Source: CAD feature listing. Evaluate the final solid. Frame: model axes, mm. A direction names the side the tool comes from. Give positions to 0.01 mm unless a question says otherwise; leave off trailing zeros. Loops run counter-clockwise (first coordinate to the right, second up) from the corner with the lowest first, then second, coordinate; pieces in that order, holes last.
```python
from build123d import *

# Parameters (mm, degrees)
SKETCH_1_R      = 2
EXTRUDE_1_DEPTH = 10


with BuildPart() as part:
    # 草图1 → 凸台-拉伸1 (new body)
    with BuildSketch(Plane.XY):
        with BuildLine():
            Line((0, 10), (-2.5, 10))
            Line((-2.5, 10), (-2.5, 27.142110135))
            Line((-2.5, 27.142110135), (-2.5, 28))
            Line((-2.5, 28), (2, 28))
            Line((2, 28), (2, 20))
            ThreePointArc((2, 20), (10, 12), (18, 20))
            Line((18, 20), (18, 28))
            Line((18, 28), (22.5, 28))
            Line((22.5, 28), (22.5, 10))
            Line((22.5, 10), (20, 10))
            Line((20, 10), (20, 0))
            Line((20, 0), (0, 0))
            Line((0, 0), (0, 10))
        make_face()
        with Locations((10, 5)):
            Circle(SKETCH_1_R, mode=Mode.SUBTRACT)
    extrude(amount=EXTRUDE_1_DEPTH)


solid = part.part
```
(1) First-contact query: pin 1 (1.5 mm diameter, centred on y = 5, z = 5.5, fed in from -X); pin 2 (8 mm diameter, centred on x = 1, y = 24.5, fed in from -Z); pin 3 (1.2 mm diameter, centred on x = -1.5, z = 5.5, fed in from -Y); pin 4 (1 mm diameter, centred on y = 8.5, z = 5, fed in from +X). Flat tips, straight axial feed; report the tip coordinate or a pass-through.
A:
pin 1: stops at x = 0
pin 2: stops at z = 0
pin 3: stops at y = 10
pin 4: stops at x = 20
(2) Section D-D, the plane y = 8.25. Return the cut outline in (x, z), then the cut area to 3 significant figures.
A:
outline: (0, 0) - (20, 0) - (20, 10) - (0, 10) - close
area: 200 mm2
(3) Section A-A, the plane x = 10. Return the cut outline in (y, z), then the cut area to 3 significant figures.
A:
outline: (0, 0) - (3, 0) - (3, 10) - (0, 10) - close; (7, 0) - (12, 0) - (12, 10) - (7, 10) - close
area: 80.0 mm2
(4) Reachability of faces 4 (the flat face through (10, 11, 0)), 5 (the flat face through (-1, 10, 5)), 6 (the flat face through (20, 5, 5)), 7 (the flat face through (18, 24, 5)), 8 (the flat face through (10, 0, 5)) from +Z, -Z, +X, -X, +Y, -Y: full face, straight path, thin tool, end or side. Return the list, or none.
A:
face 4: -Z, +X, -X, +Y, -Y
face 5: +Z, -Z, -X, -Y
face 6: +Z, -Z, +X, -Y
face 7: +Z, -Z, +Y
face 8: +Z, -Z, +X, -X, -Y
(5) Section C-C, the plane z = 1. Return the cut outline in (x, y), then the cut area to 3 significant figures.
A:
outline: (-2.5, 10) - (0, 10) - (0, 0) - (20, 0) - (20, 10) - (22.5, 10) - (22.5, 28) - (18, 28) - (18, 20) arc R8 cw to (2, 20) - (2, 28) - (-2.5, 28) - close; hole circle Ø4 at (10, 5)
area: 409 mm2
(6) Mould query, pull axis X, two halves, no side actions, for faces 1 (the cylindrical face through (10, 7, 5)), 2 (the flat face through (10, 11, 10)), 3 (the flat face through (0, 5, 5)). Classes: pulls with the +X half, pulls with the -X half, needs draft (parallel to the pull), parting line crosses it, or undercut.
A:
face 1: undercut
face 2: needs draft
face 3: pulls with the -X half
(7) Ray query, line 1 along Y through (x, z) = (10, 3.5); line 2 along X through (y, z) = (26.25, 2.25); line 3 along X through (y, z) = (1.75, 8.25). Return the intervals inside material, ascending.
A:
line 1: y = 0 to 3, 7 to 12
line 2: x = -2.5 to 2, 18 to 22.5
line 3: x = 0 to 20
(8) Section B-B, the plane y = 24.5. Return the cut outline in (x, z).
A:
outline: (-2.5, 0) - (2, 0) - (2, 10) - (-2.5, 10) - close; (18, 0) - (22.5, 0) - (22.5, 10) - (18, 10) - close
